from build123d import *

# Parameters (mm, degrees)
SKETCH1_R             = 2.5
BOSS_EXTRUDE1_DEPTH   = 12
SKETCH2_R             = 4
BOSS_EXTRUDE2_DEPTH   = 10.8
CHAMFER1_SIZE         = 0.5
CHAMFER2_SIZE         = 0.3
SKETCH3_W             = 8.000389638
SKETCH3_H             = 1
CUT_EXTRUDE1_DEPTH    = 12
M3_TAPPED_HOLE1_D     = 2.5
M3_TAPPED_HOLE1_DEPTH = 7.5
M3_TAPPED_HOLE1_TIP   = 0.751075774


with BuildPart() as part:
    # Sketch1 → Boss-Extrude1 (new body)
    with BuildSketch(Plane(origin=(0, 0, 0), x_dir=(1, 0, 0), z_dir=(0, 1, 0))):
        with Locations(Location((0, 0, 0), (0, 0, 270))):
            Circle(SKETCH1_R)
    extrude(amount=BOSS_EXTRUDE1_DEPTH)

    # Sketch2 → Boss-Extrude2 (add)
    with BuildSketch(Plane(origin=(0, 12, 0), x_dir=(1, 0, 0), z_dir=(0, 1, 0))):
        with Locations(Location((0, 0, 0), (0, 0, 90))):
            Circle(SKETCH2_R)
    extrude(amount=BOSS_EXTRUDE2_DEPTH)

    # Chamfer1
    chamfer1_edges = [part.edges().sort_by_distance(p)[0] for p in [
        (0, 12, 4),
        (0, 22.8, 4),
    ]]
    chamfer(chamfer1_edges, length=CHAMFER1_SIZE)

    # Chamfer2
    chamfer2_edges = [part.edges().sort_by_distance(p)[0] for p in [
        (0, 0, -2.5),
    ]]
    chamfer(chamfer2_edges, length=CHAMFER2_SIZE)

    # Sketch3 → Cut-Extrude1 (cut)
    with BuildSketch(Plane(origin=(0, 22.8, 0), x_dir=(1, 0, 0), z_dir=(0, 1, 0))):
        with Locations((0, 4)):
            Rectangle(SKETCH3_W, SKETCH3_H)
    extrude(amount=-CUT_EXTRUDE1_DEPTH, mode=Mode.SUBTRACT)

    # M3 Tapped Hole1
    with Locations(Plane(origin=(0, 0, 0), x_dir=(-1, 0, 0), z_dir=(0, -1, 0))):
        with Locations((0, 0)):
            Hole(M3_TAPPED_HOLE1_D / 2, depth=M3_TAPPED_HOLE1_DEPTH)
            with Locations((0, 0, -(M3_TAPPED_HOLE1_DEPTH + M3_TAPPED_HOLE1_TIP / 2))):  # 118° drill point
                Cone(0, M3_TAPPED_HOLE1_D / 2, M3_TAPPED_HOLE1_TIP, mode=Mode.SUBTRACT)


solid = part.part
Can you work these out from the model? Positions are in its coordinate system, mm. A direction names the side the tool comes from. Coordinates: 2 decimals unless noted, no trailing zeros. Loops run counter-clockwise (first coordinate to the right, second up) from the corner with the lowest first, then second, coordinate; pieces in that order, holes last. Notation, with made-up numbers: M 12,-13.75 L 23,-13.75 A29 ccw 23,10.25 Z; hole C 52.25,-21 d6. An arc over 180 degrees is marked long. Answer as CSV lines item,"result". Start each with the question number.
1. Suppose I cut it at A-A, the plane y = 18. List the corners of the cut face in (x, z) for me, plus the area to 3 significant figures.
2. For pin 1 Ø2 at (y, z) = (3, 1.5) entering from -X; pin 2 Ø1 at (x, z) = (-3, -0.5) entering from -Y, each with a flat end and sliding along its axis, tell me the tip position at first contact or that it passes through.
3. For faces 1 (the face through (2, 12, -2)), 2 (the face through (0, 22.8, 0)), which set-ups out of +Z, -Z, +X, -X, +Y, -Y let a thin tool reach every point of the face, with its end or its side?
4. Thinking about a two-plate mould opening in Z: for faces 3 (the face through (0, 17, -3.5)), 4 (the face through (0.05, 8.12, 0.21)), 5 (the face through (0, 17, 4)), 6 (the face through (-0.27, 3.8, 1.22)), which applies, +Z half, -Z half, draft (parallel to the pull), parting line (faces both ways), or undercut?
5. If I drill on probe 1 along Y at (x, z) = (1, -2.5); probe 2 along Z at (x, y) = (-0.25, 4.75); probe 3 along Z at (x, y) = (2.25, 14.5), over which ranges is the centre line in solid material (lowest first)? Write a range as [from, to].
Output:
1,outline,"M -1.94,-3.5 L 1.94,-3.5 A4 ccw long Z"
1,area,"49.0 mm^2"
2,pin 1,"stops at x = -2.45"
2,pin 2,"stops at y = 12"
3,face 1,"-Y"
3,face 2,"+Z, -Z, +X, -X, +Y"
4,face 3,"-Z half"
4,face 4,"undercut"
4,face 5,"parting line"
4,face 6,"undercut"
5,probe 1,"y = [12, 22.8]"
5,probe 2,"z = [-2.49, -1.22], [1.22, 2.49]"
5,probe 3,"z = [-3.31, 3.31]"
